Here's the drawing with two shaded views (mm, measured from the low corner). I have some questions. Coordinates: 2 decimals unless noted, no trailing zeros. Order: outer loops, then holes, each group sorted by start corner. A loop starts at its lowest first (then second) coordinate and runs counter-clockwise, first axis right, second up. Notation, with made-up numbers: (60, 11) -> (102, 11) arc R5 cw to (102, 16) -> close; hole circle Ø1 at (-14.75, 36.25). An arc over 180 degrees is marked (long way). Answer as a JSON object with one key per item and string values. Group by question number.
(1) For pin 1 (3 mm diameter, centred on y = 36, z = 5.5, fed in from -X), with a flat end and sliding along its axis, tell me the tip position at first contact or that it passes through.
(2) I want a section at A-A, the plane x = 93. List the corners of the cut face in (y, z) for me, plus the area to 3 significant figures.
(3) I need wall thicknesses on line 1 (Y direction, x = 91.5, z = 5.25); line 2 (X direction, y = 187, z = 8); line 3 (Y direction, x = 95, z = 5.25). Which ranges of each line are inside material? Lowest first, please.
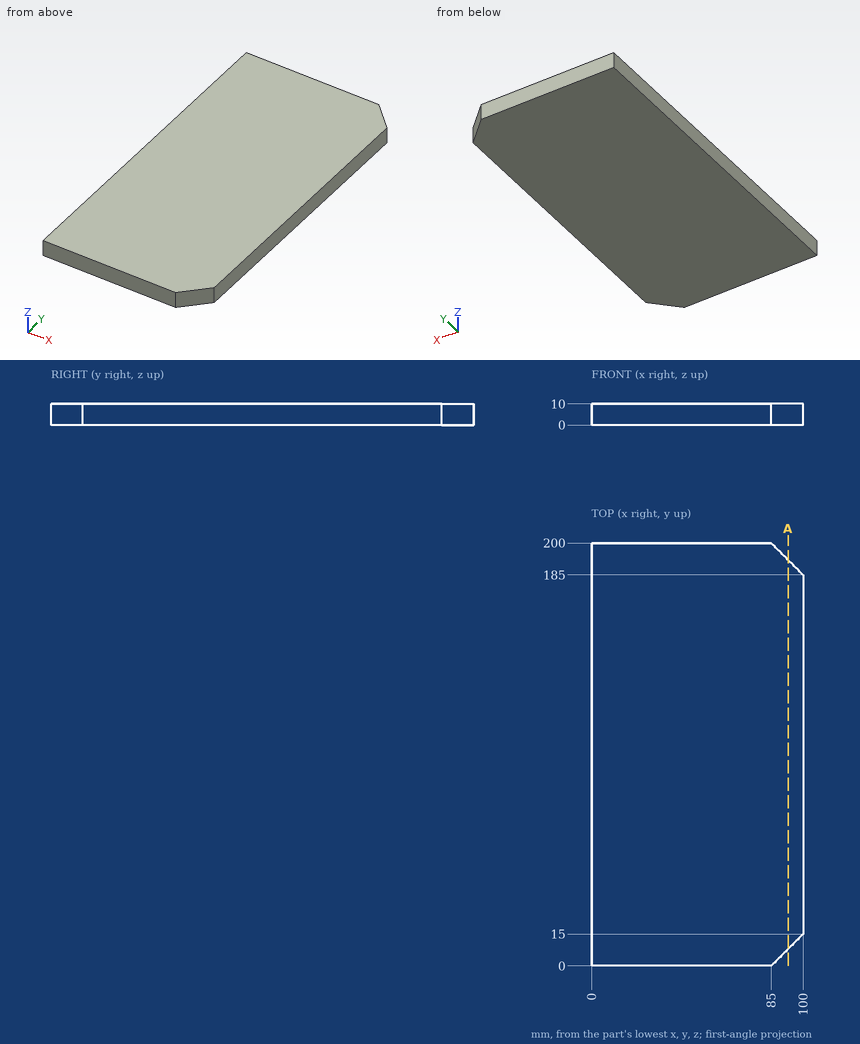
Computed values:
{
 "1": {"pin 1": "stops at x = 0"},
 "2": {"outline": "(8, 0) -> (192, 0) -> (192, 10) -> (8, 10) -> close", "area": "1,840 mm2"},
 "3": {"line 1": "y = 6.5 to 193.5", "line 2": "x = 0 to 98", "line 3": "y = 10 to 190"}
}
